from build123d import *

# Parameters (mm, degrees)
SKETCH2_R           = 127.5
CUT_EXTRUDE1_DEPTH  = 2
SKETCH3_R           = 10
BOSS_EXTRUDE1_DEPTH = 5
FILLET1_R           = 5
SKETCH4_R           = 3.15
CUT_EXTRUDE2_DEPTH  = 10
FILLET2_R           = 7.5
SKETCH5_R           = 1
CUT_EXTRUDE3_DEPTH  = 5


with BuildPart() as part:
    # Sketch1 → Revolve1 (revolve)
    with BuildSketch(Plane.XY):
        Polygon((-125, 139.5), (-125, 175.5), (-148.746139417, 175.5), (-148.746139417, 180.5), (-121, 180.5), (-121, 170.5), (-106, 170.5), (-106, 166.5), (-121, 166.5), (-121, 144.5), (-103, 144.5), (-103, 154.5), (-92, 154.5), (-92, 147.962623379), (-99, 147.962623379), (-99, 139.5), align=None)
    revolve(axis=Axis((0, 0, 0), (0, -1, 0)))

    # Sketch2 → Cut-Extrude1 (cut)
    with BuildSketch(Plane(origin=(0, 180.5, 0), x_dir=(1, 0, 0), z_dir=(0, 1, 0))):
        with Locations(Location((0, 0, 0), (0, 0, 180))):
            Circle(SKETCH2_R)
    extrude(amount=-CUT_EXTRUDE1_DEPTH, mode=Mode.SUBTRACT)

    # Sketch3 → Boss-Extrude1 (add)
    with BuildSketch(Plane.XZ.offset(-175.5)):
        with Locations((0, -148.746139417)):
            Circle(SKETCH3_R)
        with Locations((-148.746139417, 0)):
            Circle(SKETCH3_R)
        with Locations((0, 148.746139417)):
            Circle(SKETCH3_R)
        with Locations((148.746139417, 0)):
            Circle(SKETCH3_R)
    extrude(amount=-BOSS_EXTRUDE1_DEPTH)

    # Fillet1
    fillet1_edges = [part.edges().sort_by_distance(p)[0] for p in [
        (-9.994348791, 178, -148.409996239),
        (9.994348791, 178, -148.409996239),
        (-148.409996239, 178, 9.994348791),
        (-148.409996239, 178, -9.994348791),
        (9.994348791, 178, 148.409996239),
        (-9.994348791, 178, 148.409996239),
        (148.409996239, 178, -9.994348791),
        (148.409996239, 178, 9.994348791),
    ]]
    fillet(fillet1_edges, radius=FILLET1_R)

    # Sketch4 → Cut-Extrude2 (cut)
    with BuildSketch(Plane.XZ.offset(-175.5)):
        with Locations((148.746139417, 0)):
            Circle(SKETCH4_R)
        with Locations((0, -148.746139417)):
            Circle(SKETCH4_R)
        with Locations((-148.746139417, 0)):
            Circle(SKETCH4_R)
        with Locations((0, 148.746139417)):
            Circle(SKETCH4_R)
    extrude(amount=-CUT_EXTRUDE2_DEPTH, mode=Mode.SUBTRACT)

    # Fillet2
    fillet2_edges = [part.edges().sort_by_distance(p)[0] for p in [
        (125, 175.5, 0),
    ]]
    fillet(fillet2_edges, radius=FILLET2_R)

    # Sketch5 → Cut-Extrude3 (cut)
    with BuildSketch(Plane(origin=(0, 170.5, 0), x_dir=(1, 0, 0), z_dir=(0, 1, 0))):
        with Locations(Location((-116.275298476, 10, 0), (0, 0, 180))):
            Circle(SKETCH5_R)
        with Locations(Location((-116.275298476, -10, 0), (0, 0, 180))):
            Circle(SKETCH5_R)
        with Locations(Location((116.275298476, 10, 0), (0, 0, 180))):
            Circle(SKETCH5_R)
        with Locations(Location((116.275298476, -10, 0), (0, 0, 180))):
            Circle(SKETCH5_R)
    extrude(amount=-CUT_EXTRUDE3_DEPTH, mode=Mode.SUBTRACT)


solid = part.part
For this review, take the finished solid that the model builds, in its own axes (mm). A direction names the side the tool comes from. Give positions to 0.01 mm unless a question says otherwise; leave off trailing zeros. Loops run counter-clockwise (first coordinate to the right, second up) from the corner with the lowest first, then second, coordinate; pieces in that order, holes last.
Item 1: Take a section at A-A, the plane y = 160. State the section outline as (x, z) points, and give its area (3 significant figures).
Item 2: For line 1 along X through (y, z) = (152, 0); line 2 along Z through (x, y) = (0, 169), list the stretches that pass through material, from the lowest coordinate up.
Item 3: Tool access review of faces 1 (the flat face through (-71, 170.5, 80)), 2 (the flat face through (29, 147.963, 88)), 3 (the cylindrical face through (11.977, 151.186, -91.217)), 4 (the cylindrical face through (26.23, 155.346, 118.123)): name each direction out of +Z, -Z, +X, -X, +Y, -Y from which nothing blocks a thin tool from reaching the whole face with its end or side.
Item 4: Insertion check: pin 1 (4 mm diameter, centred on x = 148.75, z = 0, fed in from -Y); pin 2 (3 mm diameter, centred on x = -7, y = 169, fed in from -Z); pin 3 (10 mm diameter, centred on y = 144.5, z = -29, fed in from +X); pin 4 (3 mm diameter, centred on y = 170.5, z = -88, fed in from +X). Each pin has a flat end and moves straight along its axis. Give the tip position at first contact, or say it passes through.
Item 5: Draft analysis for pull direction X (two halves, no side actions). For faces 5 (the cylindrical face through (158.745, 177.965, -0.179)), 6 (the flat face through (-89, 144.5, -54)), 7 (the cylindrical face through (-0.179, 177.965, -158.745)), state which applies: +X half, -X half, draft (parallel to the pull), parting line (faces both ways), or undercut.
Calculated:
1. outline: circle Ø250 at (0, 0); hole circle Ø242 at (0, 0)
1. area: 3,090 mm2
2. line 1: x = -125 to -121, -103 to -92, 92 to 103, 121 to 125
2. line 2: z = -125.07 to -106, 106 to 125.07
3. face 1: +Y
3. face 2: -Y
3. face 3: +Y, -Y
3. face 4: none
4. pin 1: passes through
4. pin 2: stops at z = -125.24
4. pin 3: stops at x = 122.67
4. pin 4: stops at x = 91.08
5. face 5: +X half
5. face 6: undercut
5. face 7: parting line
